Can you work these out from the model? Positions are in its coordinate system, mm. A direction names the side the tool comes from. Coordinates: 2 decimals unless noted, no trailing zeros. Order: outer loops, then holes, each group sorted by start corner. A loop starts at its lowest first (then second) coordinate and runs counter-clockwise, first axis right, second up. Notation, with made-up numbers: M -39.75,21 L 7.25,21 A24 cw 7.25,37 Z; hole C 81,25 d2. An arc over 180 degrees is marked long. Answer as a JSON object with one key per item and string values.
from build123d import *

# Parameters (mm, degrees)
SKETCH1_R           = 18.5
SKETCH1_R_2         = 12.5
BOSS_EXTRUDE1_DEPTH = 7
SKETCH2_R           = 17.5
SKETCH2_R_2         = 13.5
CUT_EXTRUDE1_DEPTH  = 0.2
CUT_EXTRUDE2_START  = -0.2
SKETCH3_R           = 17.5
SKETCH3_R_2         = 13.5
CUT_EXTRUDE2_DEPTH  = 0.2


with BuildPart() as part:
    # Sketch1 → Boss-Extrude1 (new body)
    with BuildSketch(Plane(origin=(0, 0, 0), x_dir=(1, 0, 0), z_dir=(0, 1, 0))):
        with Locations(Location((0, 0, 0), (0, 0, 270))):
            Circle(SKETCH1_R)
        with Locations(Location((0, 0, 0), (0, 0, 270))):
            Circle(SKETCH1_R_2, mode=Mode.SUBTRACT)
    extrude(amount=BOSS_EXTRUDE1_DEPTH)

    # Sketch2 → Cut-Extrude1 (cut)
    with BuildSketch(Plane(origin=(0, 7, 0), x_dir=(1, 0, 0), z_dir=(0, 1, 0))):
        with Locations(Location((0, 0, 0), (0, 0, 270))):
            Circle(SKETCH2_R)
        with Locations(Location((0, 0, 0), (0, 0, 270))):
            Circle(SKETCH2_R_2, mode=Mode.SUBTRACT)
    extrude(amount=-CUT_EXTRUDE1_DEPTH, mode=Mode.SUBTRACT)

    # Sketch3 → Cut-Extrude2 (cut)
    with BuildSketch(Plane.XZ.offset(CUT_EXTRUDE2_START)):
        with Locations(Location((0, 0, 0), (0, 0, 90))):
            Circle(SKETCH3_R)
        with Locations(Location((0, 0, 0), (0, 0, 90))):
            Circle(SKETCH3_R_2, mode=Mode.SUBTRACT)
    extrude(amount=CUT_EXTRUDE2_DEPTH, mode=Mode.SUBTRACT)


solid = part.part
Item 1: Which directions (+Z, -Z, +X, -X, +Y, -Y) give clear straight access to the entire face, cutting with the end or side of a thin tool? Please do faces 4 (the flat face through (-14, 0, -11)), 5 (the flat face through (10.3, 0.2, 9)), 6 (the flat face through (-10.3, 6.8, 9)).
Answers follow:
{"face 4": "+Z, -Z, +X, -X, -Y", "face 5": "-Y", "face 6": "+Y"}
Item 2: I want a section at A-A, the plane x = 0. Write out the boundary of the cut face in (y, z), plus the area to 3 significant figures.
Answers follow:
{"outline": "M 0,-18.5 L 7,-18.5 L 7,-17.5 L 6.8,-17.5 L 6.8,-13.5 L 7,-13.5 L 7,-12.5 L 0,-12.5 L 0,-13.5 L 0.2,-13.5 L 0.2,-17.5 L 0,-17.5 Z; M 0,12.5 L 7,12.5 L 7,13.5 L 6.8,13.5 L 6.8,17.5 L 7,17.5 L 7,18.5 L 0,18.5 L 0,17.5 L 0.2,17.5 L 0.2,13.5 L 0,13.5 Z", "area": "80.8 mm^2"}
Item 3: If we mould it in two halves opening along Z, with no side actions, what happens to faces 1 (the cylindrical face through (3.755, 3.451, 11.923)), 2 (the cylindrical face through (-7.086, 3.451, 17.089)), 3 (the flat face through (-9, 7, 9))? For each: pulls with the +Z half, pulls with the -Z half, needs draft (parallel to the pull), parting line crosses it, or undercut.
Answers follow:
{"face 1": "undercut", "face 2": "parting line crosses it", "face 3": "needs draft"}
Item 4: I'm going to push a flat-ended pin straight in: pin 1 (1 mm diameter, centred on x = -4, y = 6, fed in from +Z). Where does the tip first touch, or does it pass through?
Answers follow:
{"pin 1": "stops at z = 18.17"}
Item 5: I want a section at D-D, the plane z = -14. Write out the boundary of the cut face in (x, y), plus the area to 3 significant figures.
Answers follow:
{"outline": "M -12.09,0 L -10.5,0 L -10.5,0.2 L 10.5,0.2 L 10.5,0 L 12.09,0 L 12.09,7 L 10.5,7 L 10.5,6.8 L -10.5,6.8 L -10.5,7 L -12.09,7 Z", "area": "161 mm^2"}
Item 6: Please list where these lines run through material, in increasing order: line 1 (X direction, y = 0.1, z = 0); line 2 (X direction, y = 2.5, z = 0); line 3 (Z direction, x = 7, y = 1.5).
Answers follow:
{"line 1": "x = -18.5 to -17.5, -13.5 to -12.5, 12.5 to 13.5, 17.5 to 18.5", "line 2": "x = -18.5 to -12.5, 12.5 to 18.5", "line 3": "z = -17.12 to -10.36, 10.36 to 17.12"}
Item 7: I want a section at C-C, the plane y = 6. Write out the boundary of the cut face in (x, z), plus the area to 3 significant figures.
Answers follow:
{"outline": "C 0,0 d37; hole C 0,0 d25", "area": "584 mm^2"}
Item 8: I want a section at B-B, the plane z = 0. Write out the boundary of the cut face in (x, y), plus the area to 3 significant figures.
Answers follow:
{"outline": "M -18.5,0 L -17.5,0 L -17.5,0.2 L -13.5,0.2 L -13.5,0 L -12.5,0 L -12.5,7 L -13.5,7 L -13.5,6.8 L -17.5,6.8 L -17.5,7 L -18.5,7 Z; M 12.5,0 L 13.5,0 L 13.5,0.2 L 17.5,0.2 L 17.5,0 L 18.5,0 L 18.5,7 L 17.5,7 L 17.5,6.8 L 13.5,6.8 L 13.5,7 L 12.5,7 Z", "area": "80.8 mm^2"}
